```python
from build123d import *

# Parameters (mm, degrees)
SKETCH_1_W         = 45
SKETCH_1_H         = 35
EXTRUDE_1_DEPTH    = 5
CHAMFER_1_SIZE     = 2
SKETCH_8_R         = 7.5
EXTRUDE_2_DEPTH    = 8.5
HOLE_WIZARD_M5_1_D = 4.2
HOLE_WIZARD_M5_2_D = 4.2


with BuildPart() as part:
    # 草图1 → 凸台-拉伸1 (new, symmetric)
    with BuildSketch(Plane(origin=(0, 0, 0), x_dir=(1, 0, 0), z_dir=(0, 1, 0))):
        Rectangle(SKETCH_1_W, SKETCH_1_H)
    extrude(amount=EXTRUDE_1_DEPTH, both=True)

    # 倒角1
    chamfer_1_edges = [part.edges().sort_by_distance(p)[0] for p in [
        (22.5, 0, 17.5),
        (-22.5, 0, 17.5),
        (-22.5, 0, -17.5),
        (22.5, 0, -17.5),
    ]]
    chamfer(chamfer_1_edges, length=CHAMFER_1_SIZE)

    # 草图8 → 凸台-拉伸2 (add)
    with BuildSketch(Plane(origin=(0, 5, 0), x_dir=(1, 0, 0), z_dir=(0, 1, 0))):
        with Locations(Location((-10, 0, 0), (0, 0, 90))):
            Circle(SKETCH_8_R)
    extrude(amount=EXTRUDE_2_DEPTH)

    # M5 螺纹孔1 (through all)
    with Locations(Plane(origin=(0, 5, 0), x_dir=(1, 0, 0), z_dir=(0, 1, 0))):
        with Locations((15, -10), (15, 10)):
            Hole(HOLE_WIZARD_M5_1_D / 2)

    # M5 螺纹孔2 (through all)
    with Locations(Plane(origin=(0, 13.5, 0), x_dir=(1, 0, 0), z_dir=(0, 1, 0))):
        with Locations((-10, 0)):
            Hole(HOLE_WIZARD_M5_2_D / 2)


solid = part.part
```
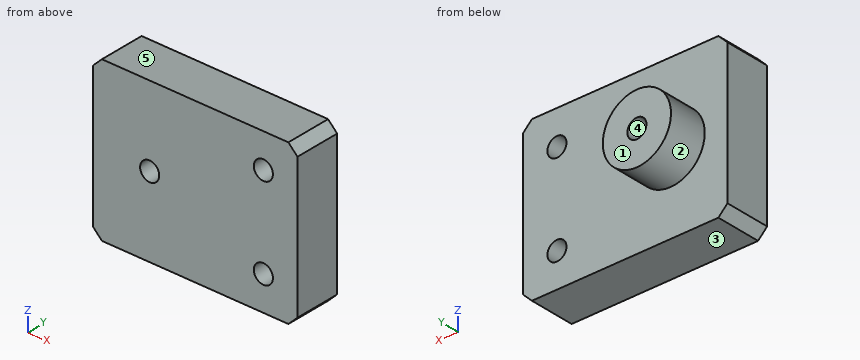
For this review, take the finished solid that the model builds, in its own axes (mm). Face numbers are marked on the shaded views. A direction names the side the tool comes from. Coordinates: 2 decimals unless noted, no trailing zeros. Loops run counter-clockwise (first coordinate to the right, second up) from the corner with the lowest first, then second, coordinate; pieces in that order, holes last. Notation, with made-up numbers: (13, -3.5) -> (56, -3.5) arc R24 cw to (56, 22.5) -> close; hole circle Ø2 at (25, 21.5). An arc over 180 degrees is marked (long way). Return JSON: item names as keys, results as strings. Group by question number.
(1) To check wall thickness, follow L1, parallel to Z at x = 15, y = -1.75; L2, parallel to X at y = -2, z = 10; L3, parallel to Y at x = -9.5, z = 8. State the ranges of each line that lie inside material, in increasing order.
(2) Consider section A-A, the plane z = -10. Give the boundary of the cut face in (x, y).
(3) Consider section D-D, the plane x = 15. Give the boundary of the cut face in (y, z), plus the area to 3 significant figures.
(4) Tool access review of the marked faces 1 and 2: name each direction out of +Z, -Z, +X, -X, +Y, -Y from which nothing blocks a thin tool from reaching the whole face with its end or side.
(5) Consider section C-C, the plane y = 1.75. Give the boundary of the cut face in (x, z).
(6) Consider section B-B, the plane x = -10. Give the boundary of the cut face in (y, z), plus the area to 3 significant figures.
(7) Mouldability with a two-part tool opening along Z and no side actions: class the marked faces 3, 4 and 5 as pulls with the +Z half, pulls with the -Z half, needs draft (parallel to the pull), parting line crosses it, or undercut.
(8) For pin 1 Ø5.5 at (x, z) = (15, -10) entering from +Y, flat-tipped, find the tip position at first contact; note if it passes through.
Results below:
{
 "1": {"L1": "z = -17.5 to -12.1, -7.9 to 7.9, 12.1 to 17.5", "L2": "x = -22.5 to 12.9, 17.1 to 22.5", "L3": "y = -5 to 5"},
 "2": {"outline": "(-22.5, -5) -> (12.9, -5) -> (12.9, 5) -> (-22.5, 5) -> close; (17.1, -5) -> (22.5, -5) -> (22.5, 5) -> (17.1, 5) -> close"},
 "3": {"outline": "(-5, -17.5) -> (5, -17.5) -> (5, -12.1) -> (-5, -12.1) -> close; (-5, -7.9) -> (5, -7.9) -> (5, 7.9) -> (-5, 7.9) -> close; (-5, 12.1) -> (5, 12.1) -> (5, 17.5) -> (-5, 17.5) -> close", "area": "266 mm2"},
 "4": {"face 1": "+Z, -Z, +X, -X, +Y", "face 2": "+Y"},
 "5": {"outline": "(-22.5, -15.5) -> (-20.5, -17.5) -> (20.5, -17.5) -> (22.5, -15.5) -> (22.5, 15.5) -> (20.5, 17.5) -> (-20.5, 17.5) -> (-22.5, 15.5) -> close; hole circle Ø4.2 at (-10, 0); hole circle Ø4.2 at (15, -10); hole circle Ø4.2 at (15, 10)"},
 "6": {"outline": "(-5, -17.5) -> (5, -17.5) -> (5, -7.5) -> (13.5, -7.5) -> (13.5, -2.1) -> (-5, -2.1) -> close; (-5, 2.1) -> (13.5, 2.1) -> (13.5, 7.5) -> (5, 7.5) -> (5, 17.5) -> (-5, 17.5) -> close", "area": "400 mm2"},
 "7": {"face 3": "pulls with the -Z half", "face 4": "undercut", "face 5": "pulls with the +Z half"},
 "8": {"pin 1": "stops at y = 5"}
}
